For this review, take the finished solid that the model builds, in its own axes (mm). A direction names the side the tool comes from. Round coordinates to 2 decimals unless told otherwise and drop trailing zeros. Order: outer loops, then holes, each group sorted by start corner. A loop starts at its lowest first (then second) coordinate and runs counter-clockwise, first axis right, second up.
from build123d import *

# Parameters (mm, degrees)
BOSS_EXTRUDE1_DEPTH = 2
SKETCH2_R           = 2.5
BOSS_EXTRUDE2_DEPTH = 7
BOSS_EXTRUDE3_DEPTH = 2
SKETCH4_R           = 2
BOSS_EXTRUDE4_DEPTH = 3
BOSS_EXTRUDE5_START = 3
SKETCH5_R           = 2
BOSS_EXTRUDE5_DEPTH = 3


with BuildPart() as part:
    # Sketch1 → Boss-Extrude1 (new body)
    with BuildSketch(Plane(origin=(0, 0, 0), x_dir=(1, 0, 0), z_dir=(0, 1, 0))):
        with BuildLine():
            Line((0, 5), (14.52, 5))
            ThreePointArc((14.52, 5), (19.52, 0), (14.52, -5))
            Line((14.52, -5), (0, -5))
            ThreePointArc((0, -5), (-5, 0), (0, 5))
        make_face()
    extrude(amount=BOSS_EXTRUDE1_DEPTH)

    # Sketch2 → Boss-Extrude2 (add)
    with BuildSketch(Plane(origin=(0, 2, 0), x_dir=(1, 0, 0), z_dir=(0, 1, 0))):
        with Locations(Location((0, 0, 0), (0, 0, 270))):
            Circle(SKETCH2_R)
        with Locations(Location((14.52, 0, 0), (0, 0, 270))):
            Circle(SKETCH2_R)
    extrude(amount=BOSS_EXTRUDE2_DEPTH)

    # Sketch3 → Boss-Extrude3 (add)
    with BuildSketch(Plane(origin=(0, 9, 0), x_dir=(1, 0, 0), z_dir=(0, 1, 0))):
        with BuildLine():
            Line((0, 5), (14.52, 5))
            ThreePointArc((14.52, 5), (19.52, 0), (14.52, -5))
            Line((14.52, -5), (0, -5))
            ThreePointArc((0, -5), (-5, 0), (0, 5))
        make_face()
    extrude(amount=BOSS_EXTRUDE3_DEPTH)

    # Sketch4 → Boss-Extrude4 (add)
    with BuildSketch(Plane(origin=(0, 11, 0), x_dir=(1, 0, 0), z_dir=(0, 1, 0))):
        with Locations(Location((0, 0, 0), (0, 0, 270))):
            Circle(SKETCH4_R)
        with Locations(Location((14.52, 0, 0), (0, 0, 270))):
            Circle(SKETCH4_R)
    extrude(amount=BOSS_EXTRUDE4_DEPTH)

    # Sketch5 → Boss-Extrude5 (add)
    with BuildSketch(Plane.XZ.offset(BOSS_EXTRUDE5_START)):
        with Locations(Location((0, 0, 0), (0, 0, 90))):
            Circle(SKETCH5_R)
        with Locations(Location((14.52, 0, 0), (0, 0, 90))):
            Circle(SKETCH5_R)
    extrude(amount=-BOSS_EXTRUDE5_DEPTH)


solid = part.part
(1) Wall thickness on L1, parallel to Y at x = 18, z = -3; L2, parallel to X at y = 12.5, z = 0; L3, parallel to Y at x = 15.5, z = -2.25: over which ranges is each line inside the solid? List them lowest first.
(2) Add section D-D on y = 3.25. Give the boundary of the cut face in (x, z).
(3) Add section A-A on z = 3. Give the boundary of the cut face in (x, y).
(4) Clearance check with flat-ended pins moving along their axes: P1, Ø5, axis at x = 6.5, z = 1, coming from the +Y side; P2, Ø3, axis at x = 3.5, z = -1.5, coming from the -Y side; P3, Ø2, axis at y = 0, z = -2, coming from the -X side. State where each tip first meets the part, or that it passes through.
(5) Tool access review of faces 1 (the face through (12.537, -1.521, -0.26)), 2 (the face through (-2, 12, 0)), 3 (the face through (17, 5.5, -0.3)): name each direction out of +Z, -Z, +X, -X, +Y, -Y from which nothing blocks a thin tool from reaching the whole face with its end or side.
(6) Draft analysis for pull direction X (two halves, no side actions). For faces 4 (the face through (15, 14, 0)), 5 (the face through (19.52, 9.99, -0.11)), 6 (the face through (7, 9, 0)), state which applies: pulls with the +X half, pulls with the -X half, needs draft (parallel to the pull), parting line crosses it, or undercut.
(7) Add section B-B on x = 7. Give the boundary of the cut face in (y, z).
Here are the results:
1. L1: y = 0 to 2, 9 to 11
1. L2: x = -2 to 2, 12.52 to 16.52
1. L3: y = 0 to 11
2. outline: circle Ø5 at (0, 0); circle Ø5 at (14.52, 0)
3. outline: (-4, 0) - (18.52, 0) - (18.52, 2) - (-4, 2) - close; (-4, 9) - (18.52, 9) - (18.52, 11) - (-4, 11) - close
4. P1: stops at y = 11
4. P2: stops at y = 0
4. P3: stops at x = -4.9
5. face 1: -Y
5. face 2: +Y
5. face 3: none
6. face 4: needs draft
6. face 5: pulls with the +X half
6. face 6: undercut
7. outline: (0, -5) - (2, -5) - (2, 5) - (0, 5) - close; (9, -5) - (11, -5) - (11, 5) - (9, 5) - close
